from build123d import *

# Parameters (mm, degrees)
BASE_PLATE_DEPTH            = 56
HUB_BOSS_SKETCH_R           = 12.5
HUB_BOSS_DEPTH              = 56
HUB_FILLET_R2_R             = 2
WEB_SKETCH_W                = 30
WEB_SKETCH_H                = 54.40435867
WEB_4MM_DEPTH               = 52
HUB_BORE_REACH              = 162.112
HUB_BORE_END_RADIUS         = 25
HUB_BORE_SKETCH_W           = 30
HUB_BORE_SKETCH_H           = 45.952641166
FLANGE_PLATE_DEPTH          = 58
FLANGE_SLOT_CUT_DEPTH       = 40
FLANGE_BOLT_HOLES_SKETCH_R  = 5
FLANGE_BOLT_HOLES_DEPTH     = 40
BASE_MOUNTING_HOLE_SKETCH_R = 8
BASE_MOUNTING_HOLE_DEPTH    = 154.738826956
FLANGE_CLOSING_BOSS_DEPTH   = 40


with BuildPart() as part:
    # Base Plate Sketch → Base Plate (new body)
    with BuildSketch(Plane.XY):
        Polygon((0, 0), (-75, 0), (-75, 18), (0, 18), (0, 27), (90, 27), (90, 0), align=None)
    extrude(amount=-BASE_PLATE_DEPTH)

    # Hub Boss Sketch → Hub Boss (add)
    with BuildSketch(Plane.XY):
        with BuildLine():
            Line((-16, 30.790627288), (-16, 18))
            Line((-16, 18), (16, 18))
            Line((16, 18), (16, 30.790627288))
            ThreePointArc((16, 30.790627288), (0, 75), (-16, 30.790627288))
        make_face()
        with Locations((0, 50)):
            Circle(HUB_BOSS_SKETCH_R, mode=Mode.SUBTRACT)
    extrude(amount=-HUB_BOSS_DEPTH)

    # Hub Fillet R2
    hub_fillet_r2_edges = [part.edges().sort_by_distance(p)[0] for p in [
        (16, 27, -28),
        (-16, 18, -28),
    ]]
    fillet(hub_fillet_r2_edges, radius=HUB_FILLET_R2_R)

    # Web Sketch → Web 4mm (add)
    with BuildSketch(Plane.XY):
        with Locations((0, 92.797820665)):
            Rectangle(WEB_SKETCH_W, WEB_SKETCH_H)
    extrude(amount=-WEB_4MM_DEPTH)

    # Hub Bore: up to this cylinder (the profile starts outside it)
    hub_bore_end = Plane(origin=(0, 50, -22.976321), z_dir=(0, 0, 1)) * Cylinder(HUB_BORE_END_RADIUS, 375.224, mode=Mode.PRIVATE)
    # Hub Bore Sketch → Hub Bore (cut, up to the surface)
    with BuildSketch(Plane(origin=(0, 120, 0), x_dir=(1, 0, 0), z_dir=(0, 1, 0)), mode=Mode.PRIVATE) as hub_bore_sk1:
        with Locations((0, 22.976320583)):
            Rectangle(HUB_BORE_SKETCH_W, HUB_BORE_SKETCH_H)
    hub_bore_tool1 = extrude(hub_bore_sk1.sketch, amount=-HUB_BORE_REACH, mode=Mode.PRIVATE) - hub_bore_end
    add(hub_bore_tool1.solids().sort_by_distance((0, 120, -22.976321))[0], mode=Mode.SUBTRACT)

    # Flange Profile Sketch → Flange Plate (add)
    with BuildSketch(Plane.XY):
        with BuildLine():
            ThreePointArc((0.584249397, 137.276236883), (-73.612691272, 99.015664074), (-79.858671486, 15.768771234))
            ThreePointArc((-79.858671486, 15.768771234), (-56.897741093, 7.377401147), (-48.506371007, 30.33833154))
            ThreePointArc((-48.506371007, 30.33833154), (-44.785464057, 79.930858496), (-0.584249397, 102.723763117))
            ThreePointArc((-0.584249397, 102.723763117), (17.276236883, 119.415750603), (0.584249397, 137.276236883))
        make_face()
    extrude(amount=-FLANGE_PLATE_DEPTH)

    # Sketch7_2 → Flange Slot Cut (cut)
    with BuildSketch(Plane.XY):
        with BuildLine():
            ThreePointArc((0.584249397, 137.276236883), (-73.612691272, 99.015664074), (-79.858671486, 15.768771234))
            ThreePointArc((-79.858671486, 15.768771234), (-56.897741093, 7.377401147), (-48.506371007, 30.33833154))
            ThreePointArc((-48.506371007, 30.33833154), (-44.785464057, 79.930858496), (-0.584249397, 102.723763117))
            ThreePointArc((-0.584249397, 102.723763117), (17.276236883, 119.415750603), (0.584249397, 137.276236883))
        make_face()
    extrude(amount=-FLANGE_SLOT_CUT_DEPTH, mode=Mode.SUBTRACT)

    # Flange Bolt Holes Sketch → Flange Bolt Holes (cut)
    with BuildSketch(Plane(origin=(0, 0, -58), x_dir=(-1, 0, 0), z_dir=(0, 0, -1))):
        with Locations((0, 120)):
            Circle(FLANGE_BOLT_HOLES_SKETCH_R)
        with Locations((39.743102788, 109.193277489)):
            Circle(FLANGE_BOLT_HOLES_SKETCH_R)
        with Locations((70.482390924, 58.635502651)):
            Circle(FLANGE_BOLT_HOLES_SKETCH_R)
        with Locations((64.182521246, 23.053551387)):
            Circle(FLANGE_BOLT_HOLES_SKETCH_R)
    extrude(amount=-FLANGE_BOLT_HOLES_DEPTH, mode=Mode.SUBTRACT)

    # Base Mounting Hole Sketch → Base Mounting Hole (cut, through all)
    with BuildSketch(Plane(origin=(0, 27, 0), x_dir=(1, 0, 0), z_dir=(0, 1, 0))):
        with Locations(Location((56, 28, 0), (0, 0, 270))):
            Circle(BASE_MOUNTING_HOLE_SKETCH_R)
        with Locations(Location((-56, 28, 0), (0, 0, 270))):
            Circle(BASE_MOUNTING_HOLE_SKETCH_R)
    extrude(amount=-BASE_MOUNTING_HOLE_DEPTH, mode=Mode.SUBTRACT)

    # Flange Closing Boss Sketch → Flange Closing Boss (add)
    with BuildSketch(Plane.XY):
        with BuildLine():
            Line((-47.651600927, 18), (-75, 18))
            Line((-75, 18), (-75, 9.570530152))
            ThreePointArc((-75, 9.570530152), (-59.090876707, 6.534324283), (-47.651600927, 18))
        make_face()
    extrude(amount=-FLANGE_CLOSING_BOSS_DEPTH)


solid = part.part
Source: CAD feature listing. Evaluate the final solid. Frame: model axes, mm. A direction names the side the tool comes from. Round coordinates to 2 decimals unless told otherwise and drop trailing zeros. Order: outer loops, then holes, each group sorted by start corner. A loop starts at its lowest first (then second) coordinate and runs counter-clockwise, first axis right, second up. Notation, with made-up numbers: (14.25, 68) -> (37.25, 68) arc R31 ccw to (37.25, 107) -> close; hole circle Ø6 at (8.5, -37.5). An arc over 180 degrees is marked (long way). Answer as CSV lines item,"result".
Item 1: Section D-D, the plane y = 120. Return loops of the section in (x, z).
A:
outline,"(-53.91, -58) -> (-5, -58) -> (-5, -40) -> (-53.91, -40) -> close; (5, -58) -> (17.29, -58) -> (17.29, -40) -> (5, -40) -> close"
Item 2: Pull-direction query (Y, two-part tool) for faces 1 (the face through (-60.215, 20.011, -49.126)), 2 (the face through (-48, 87, -58)), 3 (the face through (6, 0, -28)); classes: pulls with the +Y half, pulls with the -Y half, needs draft (parallel to the pull), parting line crosses it, or undercut.
A:
face 1,"undercut"
face 2,"needs draft"
face 3,"pulls with the -Y half"
Item 3: Section B-B, the plane x = 56. Return loops of the section in (y, z), plus the area to 3 significant figures.
A:
outline,"(0, -56) -> (27, -56) -> (27, -36) -> (0, -36) -> close; (0, -20) -> (27, -20) -> (27, 0) -> (0, 0) -> close"
area,"1,080 mm²"
Item 4: Section A-A, the plane z = -28. Return loops of the section in (x, y), plus the area to 3 significant figures.
A:
outline,"(-75, 0) -> (-64, 0) -> (-64, 5.77) arc R17.29 ccw to (-48, 16.98) -> (-48, 0) -> (48, 0) -> (48, 27) -> (18, 27) arc R2 cw to (16, 29) -> (16, 30.79) arc R25 ccw (long way) to (-16, 30.79) -> (-16, 20) arc R2 cw to (-18, 18) -> (-75, 18) -> close; (64, 0) -> (90, 0) -> (90, 27) -> (64, 27) -> close; hole circle Ø25 at (0, 50)"
area,"4,820 mm²"
Item 5: Section C-C, the plane y = 50. Return loops of the section in (x, z).
A:
outline,"(-87.8, -58) -> (-53.22, -58) -> (-53.22, -40) -> (-87.8, -40) -> close; (-25, -56) -> (-12.5, -56) -> (-12.5, 0) -> (-25, 0) -> close; (12.5, -56) -> (25, -56) -> (25, 0) -> (12.5, 0) -> close"
Item 6: Line query: L1, parallel to Y at x = 0, z = -49.5; L2, parallel to Y at x = 0, z = -44; L3, parallel to X at y = 7.5, z = -29. Output: solid intervals per line, ascending.
A:
L1,"0 to 37.5, 62.5 to 115, 125 to 137.29"
L2,"0 to 37.5, 62.5 to 75, 102.71 to 115, 125 to 137.29"
L3,"-75 to -56.64, -48.06 to 48.06, 63.94 to 90"
Item 7: Reachability of faces 4 (the face through (-16, 25, -28)), 5 (the face through (61.4, 13.7, -33.9)) from +Z, -Z, +X, -X, +Y, -Y: full face, straight path, thin tool, end or side. Return the list, or none.
A:
face 4,"+Z, -Z"
face 5,"+Y, -Y"
Item 8: Pin query (flat end, axial travel): pin 1 Ø12 at (x, z) = (-62, -21.5) entering from +Y; pin 2 Ø2 at (y, z) = (56, -49.5) entering from -X; pin 3 Ø1 at (x, y) = (-15.5, 19) entering from -Z. Return the tip coordinate at first contact, or that it passes through.
A:
pin 1,"y = 18"
pin 2,"x = -87.76"
pin 3,"z = -56"
